```python
from build123d import *

# Parameters (mm, degrees)
BOSS_EXTRUDE1_DEPTH = 1.5
BOSS_EXTRUDE3_DEPTH = 0.8
SKETCH4_R           = 1.5
CUT_EXTRUDE1_DEPTH  = 0.8
CUT_EXTRUDE2_START  = -0.5
SKETCH5_R           = 1.5
CUT_EXTRUDE2_DEPTH  = 13
SKETCH6_R           = 1.5
CUT_EXTRUDE3_DEPTH  = 7


with BuildPart() as part:
    # Sketch2 → Boss-Extrude1 (new body)
    with BuildSketch(Plane.XY):
        with BuildLine():
            Line((7.699872028, 39.883123683), (-4.438596359, 52.02159207))
            ThreePointArc((-4.438596359, 52.02159207), (-8.681237046, 52.02159207), (-8.681237046, 47.778951383))
            Line((-8.681237046, 47.778951383), (3.457231341, 35.640482996))
            ThreePointArc((3.457231341, 35.640482996), (7.699872028, 35.640482996), (7.699872028, 39.883123683))
        make_face()
    extrude(amount=BOSS_EXTRUDE1_DEPTH)

    # Sketch3 → Boss-Extrude3 (add)
    with BuildSketch(Plane.XY.offset(1.5)):
        with BuildLine():
            Line((-2.260895514, 48.429677662), (2.758792127, 43.409990022))
            ThreePointArc((2.758792127, 43.409990022), (2.758792127, 40.581562897), (-0.069634998, 40.581562897))
            Line((-0.069634998, 40.581562897), (-5.089322639, 45.601250538))
            ThreePointArc((-5.089322639, 45.601250538), (-5.089322639, 48.429677662), (-2.260895514, 48.429677662))
        make_face()
    extrude(amount=BOSS_EXTRUDE3_DEPTH)

    # Sketch4 → Cut-Extrude1 (cut)
    with BuildSketch(Plane(origin=(0, 0, 0), x_dir=(-1, 0, 0), z_dir=(0, 0, -1))):
        with Locations((-5.578551684, 37.761803339)):
            Circle(SKETCH4_R)
    extrude(amount=-CUT_EXTRUDE1_DEPTH, mode=Mode.SUBTRACT)

    # Sketch5 → Cut-Extrude2 (cut)
    with BuildSketch(Plane.XY.offset(1.5).offset(CUT_EXTRUDE2_START)):
        with Locations((-6.559916703, 49.900271726)):
            Circle(SKETCH5_R)
    extrude(amount=-CUT_EXTRUDE2_DEPTH, mode=Mode.SUBTRACT)

    # Sketch6 → Cut-Extrude3 (cut)
    with BuildSketch(Plane(origin=(0, 0, 0), x_dir=(-1, 0, 0), z_dir=(0, 0, -1))):
        with Locations((-5.578551684, 37.761803339)):
            Circle(SKETCH6_R)
    extrude(amount=-CUT_EXTRUDE3_DEPTH, mode=Mode.SUBTRACT)


solid = part.part
```
Check sheet for the modelled part. Datum: model origin and axes. Units: mm. A direction names the side the tool comes from. Coordinates: 2 decimals unless noted, no trailing zeros. Order: outer loops, then holes, each group sorted by start corner. A loop starts at its lowest first (then second) coordinate and runs counter-clockwise, first axis right, second up. Notation, with made-up numbers: M 83.25,64 L 133.25,64 A25 ccw 133.25,76 Z; hole C 55.5,3 d6. An arc over 180 degrees is marked long. Write each question's results on one line, items separated by ' | '. Start each with the question number.
1. Cross-section at C-C on y = 47.25. Record the cut outline in (x, z).
2. Cross-section at D-D on x = -4. Record the cut outline in (y, z), and give its area (3 significant figures).
3. Cross-section at B-B on y = 38.25. Record the cut outline in (x, z).
4. Cross-section at A-A on x = 6.75. Record the cut outline in (y, z), and give its area (3 significant figures).
5. Material ranges on probe 1 along Z at (x, y) = (0.25, 46); probe 2 along Y at (x, z) = (6.5, 0.8); probe 3 along Y at (x, z) = (-1.75, 0.85), recorded low to high.
6. Access from +Z, -Z, +X, -X, +Y, -Y to the whole of each face (thin tool, end or side, straight path). Record for faces 1 (the face through (-2.544, 43.056, 1.894)), 2 (the face through (-6.885, 48.436, 0.507)), 3 (the face through (-5.12, 48.4, 1.89)).
7. Mould release check, pull along X, two halves, no side actions. Record for faces 4 (the face through (-2.7, 41.8, 0.7)), 5 (the face through (5.77, 39.25, 0.74)), 6 (the face through (1.716, 45.867, 0.74)), 7 (the face through (-7, 50, 1)): +X half, -X half, draft (parallel to the pull), parting line (faces both ways), or undercut.
8. Go/stop test with flat-tipped pins: P1, Ø2.5, axis at x = -6.56, y = 49.9, coming from the -Z side; P2, Ø2.5, axis at x = 5.58, y = 37.76, coming from the +Z side. Record where each tip stops, or that it passes through.
Checks:
1) outline: M -8.15,0 L 0.33,0 L 0.33,1.5 L -1.08,1.5 L -1.08,2.3 L -5.66,2.3 L -5.66,1.5 L -8.15,1.5 Z
2) outline: M 43.1,0 L 51.58,0 L 51.58,1.5 L 48.99,1.5 L 48.99,2.3 L 44.51,2.3 L 44.51,1.5 L 43.1,1.5 Z | area: 16.3 mm²
3) outline: M 0.85,0 L 4.16,0 L 4.16,1.5 L 0.85,1.5 Z; M 7,0 L 8.54,0 L 8.54,1.5 L 7,1.5 Z
4) outline: M 35,0 L 36.82,0 L 36.82,1.5 L 35,1.5 Z; M 38.7,0 L 40.83,0 L 40.83,1.5 L 38.7,1.5 Z | area: 5.94 mm²
5) probe 1: z = 0 to 1.5 | probe 2: y = 34.91 to 36.58, 38.95 to 41.08 | probe 3: y = 40.85 to 49.33
6) face 1: +Z, -X, -Y | face 2: -Z | face 3: +Z
7) face 4: -X half | face 5: undercut | face 6: +X half | face 7: undercut
8) P1: stops at z = 1 | P2: passes through
